For this review, take the finished solid that the model builds, in its own axes (mm). A direction names the side the tool comes from. Round coordinates to 2 decimals unless told otherwise and drop trailing zeros. Write each loop counter-clockwise with the first axis right and the second up, starting at its lowest first coordinate (ties: lowest second). Pieces come first, ordered by that corner, then holes. Notation, with made-up numbers: M -33,88 L -26,88 A33 ccw -26,116 Z; hole C 50,-1.5 d1. An arc over 180 degrees is marked long. Write each question's results on one line, items separated by ' | '. Start each with the question number.
```python
from build123d import *

# Parameters (mm, degrees)
SKETCH_2_R   = 11
SKETCH_2_R_2 = 8


with BuildPart() as part:
    # Sweep 1: sweep along a path in Sketch 1
    with BuildLine(Plane.XY) as sweep_1_path:
        Line((0, 0), (15, 0))
        ThreePointArc((15, 0), (36.213203436, -8.786796564), (45, -30))
        Line((45, -30), (45, -400))
    # Sketch 2 → Sweep 1 (sweep)
    with BuildSketch(Plane(origin=(0, 0, 0), x_dir=(0, 0, -1), z_dir=(1, 0, 0))):
        Circle(SKETCH_2_R)
        Circle(SKETCH_2_R_2, mode=Mode.SUBTRACT)
    sweep(path=sweep_1_path.line)


solid = part.part
```
Item 1: We need section B-B on y = -236. State the section outline as (x, z) points.
Item 2: Insertion check: P1, Ø6, axis at y = -45.5, z = 8, coming from the -X side; P2, Ø2, axis at y = -253.5, z = 0, coming from the -X side; P3, Ø1, axis at x = 8, z = 3, coming from the +Y side. Each pin has a flat end and moves straight along its axis. Give the tip position at first contact, or say it passes through.
Item 3: For faces 1 (the flat face through (0, 8, -2)), 2 (the cylindrical face through (7.6, -10.74, 2.38)), list the 3-axis set-ups (+Z, -Z, +X, -X, +Y, -Y) from which the entire face can be reached by the end or side of a thin tool; tool diameter is ignored.
Item 4: For probe 1 along Y at (x, z) = (14.5, -1); probe 2 along X at (y, z) = (-304.5, 0); probe 3 along Y at (x, z) = (10.5, 0), list the stretches that pass through material, from the lowest coordinate up.
Item 5: We need section A-A on z = 0. State the section outline as (x, y) points, then the cut area to 3 significant figures.
Item 6: Mouldability with a two-part tool opening along Z and no side actions: class faces 3 (the cylindrical face through (55.906, -217.59, 1.432)), 4 (the cylindrical face through (52.932, -217.59, 1.041)), 5 (the flat face through (37, -400, 2)), 6 (the cylindrical face through (7.6, -7.81, 1.73)) as pulls with the +Z half, pulls with the -Z half, needs draft (parallel to the pull), parting line crosses it, or undercut.
Numbers:
1) outline: C 45,0 d22; hole C 45,0 d16
2) P1: stops at x = 35.2 | P2: stops at x = 34 | P3: stops at y = 10.71
3) face 1: +Z, -Z, -X, +Y, -Y | face 2: -X
4) probe 1: y = -10.95 to -7.94, 7.94 to 10.95 | probe 2: x = 34 to 37, 53 to 56 | probe 3: y = -11 to -8, 8 to 11
5) outline: M 0,-11 L 15,-11 A19 cw 34,-30 L 34,-400 L 37,-400 L 37,-30 A22 ccw 15,-8 L 0,-8 Z; M 0,8 L 15,8 A38 cw 53,-30 L 53,-400 L 56,-400 L 56,-30 A41 ccw 15,11 L 0,11 Z | area: 2,590 mm^2
6) face 3: parting line crosses it | face 4: undercut | face 5: needs draft | face 6: undercut
